Part model, mm, in its own coordinate system. A direction names the side the tool comes from. Round coordinates to 2 decimals unless told otherwise and drop trailing zeros. Write each question's results on one line, items separated by ' | '. Start each with the question number.
(1) Flat gauge pins, fed straight in: P1, Ø12, axis at x = 9225, y = -97.5, coming from the -Z side; P2, Ø1, axis at x = 9241, z = -35.5, coming from the -Y side; P3, Ø23.5, axis at y = 140.73, z = 68.78, coming from the +X side. Where does each tip first touch, or does it go through?
(2) Mould opens along Y. For faces 1 (the face through (9212.85, 66.63, -99.37)), 2 (the face through (9230.74, 175.72, -51.49)), 3 (the face through (9200.735, 76.4, -79.3)), 4 (the face through (9230.74, 0.396, 159.018)) say: released by +Y, released by -Y, zero draft, split by the parting line, or undercut.
(3) Drill centre lines: L1, parallel to Y at x = 9221, z = 64; L2, parallel to Y at x = 9233.5, z = -111.5; L3, parallel to X at y = 166.5, z = 14.5. Where is each one in solid material? Low to high.
(4) Cut at A-A, the plane y = 0. Give the number of separate pieces and of enclosed holes in the cut face, then the cut area to 3 significant figures.
(5) Tool access for faces 5 (the face through (9219.914, 38.887, 81.316)), 6 (the face through (9225.135, 102, -13)), 7 (the face through (9211.95, 85.19, -123.57)), 8 (the face through (9230.7, -148.7, 64.6)): list every direction of +Z, -Z, +X, -X, +Y, -Y with a clear straight run to the whole face (end or side of a thin tool).
from build123d import *

# Parameters (mm, degrees)
SKETCH2_R          = 9
CUT_EXTRUDE1_DEPTH = 267.167044388


with BuildPart() as part:
    # Sketch1 → Revolve1 (revolve)
    with BuildSketch(Plane(origin=(0, 0, 0), x_dir=(1, 0, 0), z_dir=(0, 1, 0)), mode=Mode.PRIVATE) as revolve1_sk:
        with BuildLine():
            ThreePointArc((9235.135431533, 137.473726826), (9228.064363722, 134.544794638), (9225.135431533, 127.473726826))
            Line((9225.135431533, 127.473726826), (9225.135431533, 113.473726826))
            Line((9225.135431533, 113.473726826), (9219.979100301, 113.473726826))
            Line((9219.979100301, 113.473726826), (9218.935431533, 121.973726826))
            Line((9218.935431533, 121.973726826), (9206.935431533, 121.973726826))
            Line((9206.935431533, 121.973726826), (9205.891762766, 113.473726826))
            Line((9205.891762766, 113.473726826), (9200.735431533, 113.473726826))
            Line((9200.735431533, 113.473726826), (9200.735431533, 142.473726826))
            ThreePointArc((9200.735431533, 142.473726826), (9203.664363722, 149.544794638), (9210.735431533, 152.473726826))
            Line((9210.735431533, 152.473726826), (9213.135431533, 152.473726826))
            ThreePointArc((9213.135431533, 152.473726826), (9220.206499345, 155.402659014), (9223.135431533, 162.473726826))
            Line((9223.135431533, 162.473726826), (9223.135431533, 192.473726826))
            Line((9223.135431533, 192.473726826), (9238.135431533, 192.473726826))
            Line((9238.135431533, 192.473726826), (9238.135431533, 152.473726826))
            Line((9238.135431533, 152.473726826), (9248.135431533, 152.473726826))
            Line((9248.135431533, 152.473726826), (9248.135431533, 137.473726826))
            Line((9248.135431533, 137.473726826), (9235.135431533, 137.473726826))
        make_face()
    revolve(revolve1_sk.sketch.rotate(Axis((9092.86993426, 0, -12.473726826), (1, 0, 0)), 180), axis=Axis((9092.86993426, 0, -12.473726826), (1, 0, 0)))

    # Sketch2 → Cut-Extrude1 (cut, through all)
    with BuildSketch(Plane(origin=(9238.135431533, 0, 0), x_dir=(0, 0, -1), z_dir=(1, 0, 0))):
        with Locations((-68.776273174, 140.729128115)):
            Circle(SKETCH2_R)
        with Locations((93.723726826, 140.729128115)):
            Circle(SKETCH2_R)
        with Locations((174.973726826, 0)):
            Circle(SKETCH2_R)
        with Locations((93.723726826, -140.729128115)):
            Circle(SKETCH2_R)
        with Locations((-68.776273174, -140.729128115)):
            Circle(SKETCH2_R)
        with Locations((-150.026273174, 0)):
            Circle(SKETCH2_R)
    extrude(amount=-CUT_EXTRUDE1_DEPTH, mode=Mode.SUBTRACT)


solid = part.part
A:
1) P1: z = -167.48 | P2: y = -138.18 | P3: x = 9238.14
2) face 1: undercut | face 2: split by the parting line | face 3: zero draft | face 4: undercut
3) L1: -121.81 to -65.98, 65.98 to 121.81 | L2: -150.31 to -76.06, 76.06 to 150.31 | L3: 9223.14 to 9238.14
4) separate pieces: 4 | enclosed holes: 0 | area: 3,070 mm2
5) face 5: none | face 6: +X | face 7: -X | face 8: +X, -X
